from build123d import *

# Parameters (mm, degrees)
BASE_EXTRUDE_DEPTH = 8.73125
SKETCH4_W          = 0.6
SKETCH4_H          = 11.998522628
CHAMFER_2_SIZE     = 1.4
FILLET_2_R         = 0.6


with BuildPart() as part:
    # Sketch1 → Base-Extrude (new body)
    with BuildSketch(Plane(origin=(0, 0, 0), x_dir=(0, 0, -1), z_dir=(1, 0, 0))):
        Polygon((9.525, 5.499261314), (9.525, -5.499261314), (0, -10.998522628), (-9.525, -5.499261314), (-9.525, 5.499261314), (0, 10.998522628), align=None)
    extrude(amount=BASE_EXTRUDE_DEPTH)

    # Sketch2 → Boss-Revolve1 (revolve)
    with BuildSketch(Plane.XY, mode=Mode.PRIVATE) as boss_revolve1_sk:
        Polygon((0, 0), (59.53125, 0), (59.53125, 5.55625), (59.53125, 6.35), (27.8072, 6.35), (0, 6.35), align=None)
    revolve(boss_revolve1_sk.sketch.rotate(Axis((0, 0, 0), (1, 0, 0)), 90), axis=Axis((0, 0, 0), (1, 0, 0)))

    # Sketch3 → Cut-Revolve1 (revolve, cut)
    with BuildSketch(Plane.XY, mode=Mode.PRIVATE) as cut_revolve1_sk:
        Polygon((0, 9), (4.040598923, 15.998522628), (4.040598923, 20.998522628), (-10, 20.998522628), (-10, 9), align=None)
    revolve(cut_revolve1_sk.sketch.rotate(Axis((0, 0, 0), (1, 0, 0)), 300.000000006), axis=Axis((0, 0, 0), (1, 0, 0)), mode=Mode.SUBTRACT)

    # Sketch5 → Cut-Revolve2 (revolve, cut)
    with BuildSketch(Plane.XY, mode=Mode.PRIVATE) as cut_revolve2_sk:
        Polygon((8.73125, 9), (4.690651077, 15.998522628), (4.690651077, 20.998522628), (14.690651077, 20.998522628), (14.690651077, 9), align=None)
    revolve(cut_revolve2_sk.sketch.rotate(Axis((0, 0, 0), (1, 0, 0)), 90), axis=Axis((0, 0, 0), (1, 0, 0)), mode=Mode.SUBTRACT)

    # Sketch4 → Cut-Revolve3 (revolve, cut)
    with BuildSketch(Plane.XY, mode=Mode.PRIVATE) as cut_revolve3_sk:
        with Locations((8.43125, 14.999261314)):
            Rectangle(SKETCH4_W, SKETCH4_H)
    revolve(cut_revolve3_sk.sketch.rotate(Axis((0, 0, 0), (1, 0, 0)), 90), axis=Axis((0, 0, 0), (1, 0, 0)), mode=Mode.SUBTRACT)

    # Chamfer 2
    chamfer_2_edges = [part.edges().sort_by_distance(p)[0] for p in [
        (59.53125, 0, -6.35),
    ]]
    chamfer(chamfer_2_edges, length=CHAMFER_2_SIZE)

    # Fillet 2
    fillet_2_edges = [part.edges().sort_by_distance(p)[0] for p in [
        (8.73125, 0, -6.35),
    ]]
    fillet(fillet_2_edges, radius=FILLET_2_R)


solid = part.part
Can you work these out from the model? Positions are in its coordinate system, mm. A direction names the side the tool comes from. Give positions to 0.01 mm unless a question says otherwise; leave off trailing zeros. Loops run counter-clockwise (first coordinate to the right, second up) from the corner with the lowest first, then second, coordinate; pieces in that order, holes last. Notation, with made-up numbers: (-1, 47.5) - (28, 47.5) arc R18 cw to (28, 56.5) - close; hole circle Ø8 at (72, 49.5). An arc over 180 degrees is marked (long way). One line per item, written item: value.
(1) On a 3-axis mill with a long thin cutter (end or side, diameter ignored), from which of +Z, -Z, +X, -X, +Y, -Y can I reach the whole of each face in a straight line? I mean faces 1 (the face through (7.97, -5.18, -8.92)), 2 (the face through (33.39, 3.86, -5.04)). Say none if no direction works.
Verdict:
face 1: -Z, +X, -Y
face 2: +X
(2) If we section it at C-C, the plane x = 28.5: List the corners of the cut face in (y, z) for me, plus the area to 3 significant figures.
Verdict:
outline: circle Ø12.7 at (0, 0)
area: 127 mm^2
(3) I'm going to push flat-ended pins straight in: pin 1 (1 mm diameter, centred on x = 11.5, z = -3, fed in from -Y); pin 2 (4 mm diameter, centred on x = 13, y = -7, fed in from -Z); pin 3 (4 mm diameter, centred on x = 9.5, z = -7, fed in from -Y); pin 4 (9 mm diameter, centred on y = 4, z = 4, fed in from +X). Where does each tip first touch, or does it pass through?
Verdict:
pin 1: y = -5.84
pin 2: z = -3.91
pin 3: y = -7.8
pin 4: x = 59.53
(4) If we section it at B-B, the plane x = 6.5: List the corners of the cut face in (y, z) for me (3 decimals), plus the area to 3 significant figures.
Verdict:
outline: (-10.999, 0) - (-5.499, -9.525) - (5.499, -9.525) - (10.999, 0) - (5.499, 9.525) - (-5.499, 9.525) - close
area: 314 mm^2
(5) If we section it at A-A, the plane y = 0: List the corners of the cut face in (x, z) for me (3 decimals), plus the area to 3 significant figures.
Verdict:
outline: (0, -9) - (0.303, -9.525) - (8.131, -9.525) - (8.131, -9) - (8.731, -9) - (8.731, -6.95) arc R0.6 cw to (9.331, -6.35) - (58.131, -6.35) - (59.531, -4.95) - (59.531, 4.95) - (58.131, 6.35) - (9.331, 6.35) arc R0.6 cw to (8.731, 6.95) - (8.731, 9) - (8.131, 9) - (8.131, 9.525) - (0.303, 9.525) - (0, 9) - close
area: 809 mm^2
(6) I need wall thicknesses on line 1 along X through (y, z) = (6.75, 2); line 2 along Y through (x, z) = (40, -5.5); line 3 along Z through (x, y) = (49.5, -5). Which ranges of each line are inside material? Lowest first, please.
Verdict:
line 1: 0 to 8.73
line 2: -3.17 to 3.17
line 3: -3.91 to 3.91
